Work out the finished part from the listing and answer in its coordinate system (mm). Face numbers are marked on the shaded views. Coordinates: 2 decimals unless noted, no trailing zeros. Loops run counter-clockwise (first coordinate to the right, second up) from the corner with the lowest first, then second, coordinate; pieces in that order, holes last. Notation, with made-up numbers: (59, 64.25) -> (75, 64.25) arc R7 cw to (75, 71.25) -> close; hole circle Ø8 at (55.25, -36). An arc over 180 degrees is marked (long way). Answer as CSV lines item,"result".
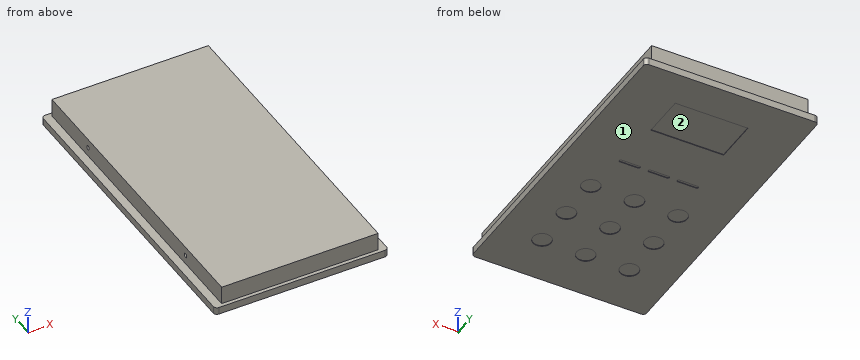
```python
from build123d import *

# Parameters (mm, degrees)
EXTRUDE_1_DEPTH          = 10
SKETCH_2_W               = 215
SKETCH_2_H               = 418
EXTRUDE_2_DEPTH          = 25
CUT_EXTRUDE_1_DEPTH      = 314.565383931
CUT_EXTRUDE_1_DEPTH_BACK = 314.565383931
SKETCH_3_R               = 3
SKETCH_4_R               = 12.5
SKETCH_4_W               = 100
SKETCH_4_H               = 60
CUT_EXTRUDE_2_DEPTH      = 1


with BuildPart() as part:
    # 草图1 → 凸台-拉伸1 (new body)
    with BuildSketch(Plane.XY):
        with BuildLine():
            Line((-114, 214), (114, 214))
            ThreePointArc((114, 214), (117.535533906, 212.535533906), (119, 209))
            Line((119, 209), (119, -209))
            ThreePointArc((119, -209), (117.535533906, -212.535533906), (114, -214))
            Line((114, -214), (-114, -214))
            ThreePointArc((-114, -214), (-117.535533906, -212.535533906), (-119, -209))
            Line((-119, -209), (-119, 209))
            ThreePointArc((-119, 209), (-117.535533906, 212.535533906), (-114, 214))
        make_face()
    extrude(amount=EXTRUDE_1_DEPTH)

    # 草图2 → 凸台-拉伸2 (add)
    with BuildSketch(Plane.XY.offset(10)):
        Rectangle(SKETCH_2_W, SKETCH_2_H)
    extrude(amount=EXTRUDE_2_DEPTH)

    # 草图3 → 切除-拉伸1 (cut, two sides: drawn at the far end of the back side and taken through both)
    with BuildSketch(Plane(origin=(107.5, 0, 0), x_dir=(0, 0, -1), z_dir=(1, 0, 0)).offset(-CUT_EXTRUDE_1_DEPTH_BACK)):
        with Locations(Location((-22.5, 120, 0), (0, 0, 90))):
            Circle(SKETCH_3_R)
        with Locations(Location((-22.5, -120, 0), (0, 0, 90))):
            Circle(SKETCH_3_R)
    extrude(amount=CUT_EXTRUDE_1_DEPTH + CUT_EXTRUDE_1_DEPTH_BACK, mode=Mode.SUBTRACT)

    # 草图4 → 切除-拉伸2 (cut)
    with BuildSketch(Plane(origin=(0, 0, 0), x_dir=(-1, 0, 0), z_dir=(0, 0, -1))):
        with Locations((0, -26)):
            Circle(SKETCH_4_R)
        with Locations((60, -26)):
            Circle(SKETCH_4_R)
        with Locations((60, -86)):
            Circle(SKETCH_4_R)
        with Locations((60, -146)):
            Circle(SKETCH_4_R)
        with Locations((0, -86)):
            Circle(SKETCH_4_R)
        with Locations((0, -146)):
            Circle(SKETCH_4_R)
        with Locations(Location((-60, -146, 0), (0, 0, 180))):
            Circle(SKETCH_4_R)
        with Locations(Location((-60, -86, 0), (0, 0, 180))):
            Circle(SKETCH_4_R)
        with Locations(Location((-60, -26, 0), (0, 0, 180))):
            Circle(SKETCH_4_R)
        with Locations((0, 134)):
            Rectangle(SKETCH_4_W, SKETCH_4_H)
        with BuildLine():
            Line((-12.5, 36), (12.5, 36))
            ThreePointArc((12.5, 36), (14.5, 34), (12.5, 32))
            Line((12.5, 32), (-12.5, 32))
            ThreePointArc((-12.5, 32), (-14.5, 34), (-12.5, 36))
        make_face()
        with BuildLine():
            Line((27.5, 36), (52.5, 36))
            ThreePointArc((52.5, 36), (54.5, 34), (52.5, 32))
            Line((52.5, 32), (27.5, 32))
            ThreePointArc((27.5, 32), (25.5, 34), (27.5, 36))
        make_face()
        with BuildLine():
            Line((-27.5, 36), (-52.5, 36))
            ThreePointArc((-52.5, 36), (-54.5, 34), (-52.5, 32))
            Line((-52.5, 32), (-27.5, 32))
            ThreePointArc((-27.5, 32), (-25.5, 34), (-27.5, 36))
        make_face()
    extrude(amount=-CUT_EXTRUDE_2_DEPTH, mode=Mode.SUBTRACT)


solid = part.part
```
(1) For a pull along X with two mould halves and no side action, classify the marked faces 1 and 2 as pulls with the +X half, pulls with the -X half, needs draft (parallel to the pull), parting line crosses it, or undercut.
Computed values:
face 1,"needs draft"
face 2,"undercut"
(2) Flat-ended cylindrical pins translate along their axes: pin 1 Ø8 at (x, z) = (44.5, 18) entering from +Y; pin 2 Ø8 at (x, z) = (88, 12.5) entering from -Y; pin 3 Ø12.5 at (x, y) = (0, -24.5) entering from -Z; pin 4 Ø12.5 at (y, z) = (27.5, 19) entering from -X. Find the tip coordinate at first contact, or state that the pin passes through.
Computed values:
pin 1,"y = 209"
pin 2,"y = -214"
pin 3,"z = 1"
pin 4,"x = -107.5"
(3) A cutting plane is placed at D-D, the plane z = 14.5. Write down the section's boundary in (x, y).
Computed values:
outline,"(-107.5, -209) -> (107.5, -209) -> (107.5, 209) -> (-107.5, 209) -> close"
(4) Consider line 1 along Y through (x, z) = (0, 0.6); line 2 along Y through (x, z) = (3, 22); line 3 along Y through (x, z) = (-60, 0.7). Determine where each line is inside the solid, lowest interval first.
Computed values:
line 1,"-214 to -158.5, -133.5 to -98.5, -73.5 to -38.5, -13.5 to 32, 36 to 104, 164 to 214"
line 2,"-209 to -122.96, -117.04 to 117.04, 122.96 to 209"
line 3,"-214 to -158.5, -133.5 to -98.5, -73.5 to -38.5, -13.5 to 214"
(5) A cutting plane is placed at B-B, the plane y = -146. Write down the section's boundary in (x, z), and give its area (3 significant figures).
Computed values:
outline,"(-119, 0) -> (-72.5, 0) -> (-72.5, 1) -> (-47.5, 1) -> (-47.5, 0) -> (-12.5, 0) -> (-12.5, 1) -> (12.5, 1) -> (12.5, 0) -> (47.5, 0) -> (47.5, 1) -> (72.5, 1) -> (72.5, 0) -> (119, 0) -> (119, 10) -> (107.5, 10) -> (107.5, 35) -> (-107.5, 35) -> (-107.5, 10) -> (-119, 10) -> close"
area,"7,680 mm2"
(6) A cutting plane is placed at A-A, the plane x = -60. Write down the section's boundary in (y, z).
Computed values:
outline,"(-214, 0) -> (-158.5, 0) -> (-158.5, 1) -> (-133.5, 1) -> (-133.5, 0) -> (-98.5, 0) -> (-98.5, 1) -> (-73.5, 1) -> (-73.5, 0) -> (-38.5, 0) -> (-38.5, 1) -> (-13.5, 1) -> (-13.5, 0) -> (214, 0) -> (214, 10) -> (209, 10) -> (209, 35) -> (-209, 35) -> (-209, 10) -> (-214, 10) -> close; hole circle Ø6 at (-120, 22.5); hole circle Ø6 at (120, 22.5)"
(7) A cutting plane is placed at C-C, the plane x = 35. Write down the section's boundary in (y, z).
Computed values:
outline,"(-214, 0) -> (32, 0) -> (32, 1) -> (36, 1) -> (36, 0) -> (104, 0) -> (104, 1) -> (164, 1) -> (164, 0) -> (214, 0) -> (214, 10) -> (209, 10) -> (209, 35) -> (-209, 35) -> (-209, 10) -> (-214, 10) -> close; hole circle Ø6 at (-120, 22.5); hole circle Ø6 at (120, 22.5)"
